Read the model definition and answer for the solid it produces. Units are mm, in the model's axes. A direction names the side the tool comes from. Give positions to 0.01 mm unless a question says otherwise; leave off trailing zeros. Order: outer loops, then holes, each group sorted by start corner. A loop starts at its lowest first (then second) coordinate and runs counter-clockwise, first axis right, second up. Notation, with made-up numbers: (-36, -8.5) - (-26, -8.5) arc R7 cw to (-26, 0.5) - close; hole circle Ø9 at (52, 85). An arc over 180 degrees is marked (long way). Answer as CSV lines item,"result". Start each with the question number.
from build123d import *

# Parameters (mm, degrees)
SKETCH2_R = 2.5


with BuildPart() as part:
    # Sweep1: sweep along a path in Sketch1
    with BuildLine(Plane(origin=(0, 0, 0), x_dir=(1, 0, 0), z_dir=(0, 1, 0))) as sweep1_path:
        Line((0, 0), (-20, 0))
        ThreePointArc((-20, 0), (-34.142135624, -5.857864376), (-40, -20))
        Line((-40, -20), (-40, -60))
        ThreePointArc((-40, -60), (-34.142135624, -74.142135624), (-20, -80))
        Line((-20, -80), (0, -80))
    # Sketch2 → Sweep1 (sweep)
    with BuildSketch(Plane(origin=(0, 0, 0), x_dir=(0, 0, -1), z_dir=(1, 0, 0))):
        Circle(SKETCH2_R)
    sweep(path=sweep1_path.line)


solid = part.part
(1) Straight lines are drawn through the part: line 1 (X direction, y = -0.25, z = 22.5); line 2 (Z direction, x = -25.5, y = 0.4); line 3 (Z direction, x = -10, y = 2.2). For each, find the intervals that lie inside material, in ascending order. Write a range as [from, to].
(2) Determine the mould class of faces 4 (the cylindrical face through (-10.14, 2.44, 0.54)), 5 (the flat face through (0, 0, 80)) for opening direction Z: released by +Z, released by -Z, zero draft, split by the parting line, or undercut.
(3) Flat-ended cylindrical pins translate along their axes: pin 1 Ø1.5 at (x, y) = (-25.5, -0.5) entering from -Z; pin 2 Ø3 at (y, z) = (2, 40) entering from -X; pin 3 Ø2 at (x, y) = (-29, -1) entering from +Z. Find the tip coordinate at first contact, or state that the pin passes through.
(4) Section B-B, the plane x = -8 is taken. Write down the section's boundary in (y, z), and give its area (3 significant figures).
(5) Which of the six approach directions +Z, -Z, +X, -X, +Y, -Y give full straight-line access (tool end or side, diameter ignored) to faces 1 (the flat face through (0, 0, 0)), 2 (the cylindrical face through (-9.9, -0.1, 77.5)), 3 (the cylindrical face through (-42.31, 0.96, 40.28))?
(6) Section C-C, the plane z = 50 is taken. Write down the section's boundary in (x, y), and give its area (3 significant figures).
(7) Section A-A, the plane y = 0 is taken. Write down the section's boundary in (x, z).
Checks:
1,line 1,"x = [-42.49, -37.51]"
1,line 2,"z = [-1.78, 3.35], [76.65, 81.78]"
1,line 3,"z = [-1.19, 1.19], [78.81, 81.19]"
2,face 4,"undercut"
2,face 5,"zero draft"
3,pin 1,"stops at z = -1.97"
3,pin 2,"stops at x = -42.45"
3,pin 3,"stops at z = 80.92"
4,outline,"circle Ø5 at (0, 0); circle Ø5 at (0, 80)"
4,area,"39.3 mm²"
5,face 1,"+Z, -Z, +X, +Y, -Y"
5,face 2,"+X"
5,face 3,"none"
6,outline,"circle Ø5 at (-40, 0)"
6,area,"19.6 mm²"
7,outline,"(-42.5, 20) arc R22.5 ccw to (-20, -2.5) - (0, -2.5) - (0, 2.5) - (-20, 2.5) arc R17.5 cw to (-37.5, 20) - (-37.5, 60) arc R17.5 cw to (-20, 77.5) - (0, 77.5) - (0, 82.5) - (-20, 82.5) arc R22.5 ccw to (-42.5, 60) - close"
